```python
from build123d import *

# Parameters (mm, degrees)
BOSS_EXTRUDE1_DEPTH = 5
SKETCH2_W           = 20
SKETCH2_H           = 160
CUT_EXTRUDE1_DEPTH  = 10


with BuildPart() as part:
    # Sketch1 → Boss-Extrude1 (new, symmetric)
    with BuildSketch(Plane.XY):
        with BuildLine():
            Line((-30, 203.803827246), (-30, 30))
            Line((-30, 30), (20, 30))
            Line((20, 30), (20, 40))
            Line((20, 40), (56.500321431, 198.100261681))
            ThreePointArc((56.500321431, 198.100261681), (13.55357606, 205.553644035), (-30, 203.803827246))
        make_face()
    extrude(amount=BOSS_EXTRUDE1_DEPTH, both=True)

    # Sketch2 → Cut-Extrude1 (cut)
    with BuildSketch(Plane.XY.offset(5)):
        with Locations((0, 30)):
            Rectangle(SKETCH2_W, SKETCH2_H)
    extrude(amount=-CUT_EXTRUDE1_DEPTH, mode=Mode.SUBTRACT)


solid = part.part
```
CAD build for the part. Positions are in the model's coordinates, mm. A direction names the side the tool comes from. Coordinates: 2 decimals unless noted, no trailing zeros. Write each loop counter-clockwise with the first axis right and the second up, starting at its lowest first coordinate (ties: lowest second). Pieces come first, ordered by that corner, then holes. Notation, with made-up numbers: (-15, 18.5) -> (36, 18.5) arc R24 cw to (36, 52.5) -> close; hole circle Ø5 at (12, 72). An arc over 180 degrees is marked (long way). Use CSV: the item, a comma, the result in double quotes. Start each with the question number.
Item 1: Two-plate mould, pull along X, no slides. Class faces 1 (the flat face through (10, 69, 0)), 2 (the flat face through (15, 30, 0)), 3 (the flat face through (20, 35, 0)): +X half, -X half, draft (parallel to the pull), parting line (faces both ways), or undercut.
Item 2: Tool access for faces 4 (the flat face through (-10, 69, 0)), 5 (the flat face through (-20, 30, 0)): list every direction of +Z, -Z, +X, -X, +Y, -Y with a clear straight run to the whole face (end or side of a thin tool).
Item 3: Band-saw the part on C-C, the plane y = 46.5. Write the cut outline in (x, z).
Item 4: Band-saw the part on D-D, the plane x = -7.5. Write the cut outline in (y, z), plus the area to 3 significant figures.
Item 5: Band-saw the part on B-B, the plane y = 81. Write the cut outline in (x, z), plus the area to 3 significant figures.
Item 6: Wall check: probe 1 along X at (y, z) = (76.5, -0.25); probe 2 along X at (y, z) = (46, -1); probe 3 along X at (y, z) = (151.5, -0.25). Give the ranges that are in metal, low to high.
Item 7: Band-saw the part on A-A, the plane z = 2.75. Write the cut outline in (x, y).
Item 8: Drop flat-ended pins along their axis: P1, Ø6, axis at x = 46.5, z = 3.5, coming from the +Y side; P2, Ø5, axis at x = 0, z = 2, coming from the -Y side. Give the stop position or say it passes through.
Response values:
1,face 1,"undercut"
1,face 2,"draft"
1,face 3,"+X half"
2,face 4,"+Z, -Z, -Y"
2,face 5,"+Z, -Z, +X, -X, -Y"
3,outline,"(-30, -5) -> (-10, -5) -> (-10, 5) -> (-30, 5) -> close; (10, -5) -> (21.5, -5) -> (21.5, 5) -> (10, 5) -> close"
4,outline,"(110, -5) -> (205.86, -5) -> (205.86, 5) -> (110, 5) -> close"
4,area,"959 mm2"
5,outline,"(-30, -5) -> (-10, -5) -> (-10, 5) -> (-30, 5) -> close; (10, -5) -> (29.47, -5) -> (29.47, 5) -> (10, 5) -> close"
5,area,"395 mm2"
6,probe 1,"x = -30 to -10, 10 to 28.43"
6,probe 2,"x = -30 to -10, 10 to 21.39"
6,probe 3,"x = -30 to 45.74"
7,outline,"(-30, 30) -> (-10, 30) -> (-10, 110) -> (10, 110) -> (10, 30) -> (20, 30) -> (20, 40) -> (56.5, 198.1) arc R206 ccw to (-30, 203.8) -> close"
8,P1,"stops at y = 201.35"
8,P2,"stops at y = 110"
